CAD build for the part. Positions are in the model's coordinates, mm. A direction names the side the tool comes from. Round coordinates to 2 decimals unless told otherwise and drop trailing zeros. Write each loop counter-clockwise with the first axis right and the second up, starting at its lowest first coordinate (ties: lowest second). Pieces come first, ordered by that corner, then holes. Notation, with made-up numbers: (-6.5, 60) -> (35.5, 60) arc R19 cw to (35.5, 94) -> close; hole circle Ø3 at (12.25, 76). An arc over 180 degrees is marked (long way). Put each result on its own line as item: value. Start each with the question number.
1. Saw through at D-D on x = -4. List the corners of the cut face in (y, z).
2. Flat gauge pins, fed straight in: P1, Ø8, axis at x = -33, y = 33, coming from the -Z side; P2, Ø3, axis at x = 20.5, z = -17.5, coming from the -Y side; P3, Ø12, axis at x = -2.5, y = 25.5, coming from the +Z side. Where does each tip first touch, or does it go through?
3. Saw through at A-A on z = -10.75. List the corners of the cut face in (x, y).
4. Pull direction Z, two halves, no side cores. Call faces 1 (the flat face through (-24, 8, -17)), 2 (the flat face through (30, 32, -2.5)), 3 (the cylindrical face through (23.846, 7.509, -20.944)): pulls with the +Z half, pulls with the -Z half, needs draft (parallel to the pull), parting line crosses it, or undercut.
5. Saw through at C-C on x = -32. State how many separate pieces and enclosed holes the cut face has, and give its area (3 significant figures).
6. 3-axis set-ups, long thin cutter, end or side, ignore diameter. For faces 4 (the flat face through (30, -35, -2.5)), 5 (the flat face through (-31, 30, -22.5)), 6 (the flat face through (30, 32, -22.5)), 7 (the cylindrical face through (-30.237, -29.866, -12.36)): which of +Z, -Z, +X, -X, +Y, -Y reach the whole face in a straight line?
7. Saw through at B-B on y = 10. List the corners of the cut face in (x, z).
8. Drill centre lines: line 1 (Y direction, x = -33, z = -23.1); line 2 (Z direction, x = 36, y = 28). Where is each one in solid material? Low to high. Write a range as from..to.
from build123d import *

# Parameters (mm, degrees)
FRONT_FLANGE_80X80_DEPTH = 2.5
HOUSING_BODY_DEPTH       = 20
REAR_FLANGE_80X80_DEPTH  = 2.5
MOUNTING_HOLES_SKETCH_R  = 3
MOUNTING_HOLES_4X_DEPTH  = 92.5
THROUGH_BORE_SKETCH_50_R = 25
THROUGH_BORE_50_DEPTH    = 132.5
COUNTERBORE_SKETCH_70_R  = 35
COUNTERBORE_70_DEPTH     = 17


with BuildPart() as part:
    # Front Flange Sketch → Front Flange 80x80 (new body)
    with BuildSketch(Plane.XY):
        with BuildLine():
            Line((-33, -40), (33, -40))
            ThreePointArc((33, -40), (37.949747468, -37.949747468), (40, -33))
            Line((40, -33), (40, 33))
            ThreePointArc((40, 33), (37.949747468, 37.949747468), (33, 40))
            Line((33, 40), (-33, 40))
            ThreePointArc((-33, 40), (-37.949747468, 37.949747468), (-40, 33))
            Line((-40, 33), (-40, -33))
            ThreePointArc((-40, -33), (-37.949747468, -37.949747468), (-33, -40))
        make_face()
    extrude(amount=-FRONT_FLANGE_80X80_DEPTH)

    # Housing Body Sketch → Housing Body (add)
    with BuildSketch(Plane(origin=(0, 0, -2.5), x_dir=(-1, 0, 0), z_dir=(0, 0, -1))):
        with BuildLine():
            Line((-14.361406616, 40), (14.361406616, 40))
            ThreePointArc((14.361406616, 40), (30.0520382, 30.0520382), (40, 14.361406616))
            Line((40, 14.361406616), (40, -14.361406616))
            ThreePointArc((40, -14.361406616), (30.0520382, -30.0520382), (14.361406616, -40))
            Line((14.361406616, -40), (-14.361406616, -40))
            ThreePointArc((-14.361406616, -40), (-30.0520382, -30.0520382), (-40, -14.361406616))
            Line((-40, -14.361406616), (-40, 14.361406616))
            ThreePointArc((-40, 14.361406616), (-30.0520382, 30.0520382), (-14.361406616, 40))
        make_face()
    extrude(amount=HOUSING_BODY_DEPTH)

    # Rear Flange Sketch → Rear Flange 80x80 (add)
    with BuildSketch(Plane(origin=(0, 0, -22.5), x_dir=(-1, 0, 0), z_dir=(0, 0, -1))):
        with BuildLine():
            Line((33, -40), (-33, -40))
            ThreePointArc((-33, -40), (-37.949747468, -37.949747468), (-40, -33))
            Line((-40, -33), (-40, 33))
            ThreePointArc((-40, 33), (-37.949747468, 37.949747468), (-33, 40))
            Line((-33, 40), (33, 40))
            ThreePointArc((33, 40), (37.949747468, 37.949747468), (40, 33))
            Line((40, 33), (40, -33))
            ThreePointArc((40, -33), (37.949747468, -37.949747468), (33, -40))
        make_face()
    extrude(amount=REAR_FLANGE_80X80_DEPTH)

    # Mounting Holes Sketch → Mounting Holes 4x (cut)
    with BuildSketch(Plane.XY):
        with Locations(Location((-33, 33, 0), (0, 0, 180))):
            Circle(MOUNTING_HOLES_SKETCH_R)
        with Locations(Location((33, 33, 0), (0, 0, 180))):
            Circle(MOUNTING_HOLES_SKETCH_R)
        with Locations(Location((33, -33, 0), (0, 0, 180))):
            Circle(MOUNTING_HOLES_SKETCH_R)
        with Locations(Location((-33, -33, 0), (0, 0, 180))):
            Circle(MOUNTING_HOLES_SKETCH_R)
    extrude(amount=-MOUNTING_HOLES_4X_DEPTH, mode=Mode.SUBTRACT)

    # Through Bore Sketch Ø50 → Through Bore Ø50 (cut)
    with BuildSketch(Plane.XY):
        Circle(THROUGH_BORE_SKETCH_50_R)
    extrude(amount=-THROUGH_BORE_50_DEPTH, mode=Mode.SUBTRACT)

    # Counterbore Sketch Ø70 → Counterbore Ø70 (cut)
    with BuildSketch(Plane.XY):
        Circle(COUNTERBORE_SKETCH_70_R)
    extrude(amount=-COUNTERBORE_70_DEPTH, mode=Mode.SUBTRACT)


solid = part.part
Return value:
1. outline: (-40, -25) -> (-24.68, -25) -> (-24.68, -17) -> (-34.77, -17) -> (-34.77, 0) -> (-40, 0) -> close; (24.68, -25) -> (40, -25) -> (40, 0) -> (34.77, 0) -> (34.77, -17) -> (24.68, -17) -> close
2. P1: stops at z = -25
2. P2: stops at y = -38.02
2. P3: stops at z = -17
3. outline: (-40, -14.36) arc R42.5 ccw to (-14.36, -40) -> (14.36, -40) arc R42.5 ccw to (40, -14.36) -> (40, 14.36) arc R42.5 ccw to (14.36, 40) -> (-14.36, 40) arc R42.5 ccw to (-40, 14.36) -> close; hole circle Ø70 at (0, 0)
4. face 1: pulls with the +Z half
4. face 2: undercut
4. face 3: needs draft
5. separate pieces: 5
5. enclosed holes: 0
5. area: 980 mm^2
6. face 4: +X, -Y
6. face 5: -X, +Y
6. face 6: +X, +Y
6. face 7: -X, -Y
7. outline: (-40, -25) -> (-22.91, -25) -> (-22.91, -17) -> (-33.54, -17) -> (-33.54, 0) -> (-40, 0) -> close; (22.91, -25) -> (40, -25) -> (40, 0) -> (33.54, 0) -> (33.54, -17) -> (22.91, -17) -> close
8. line 1: y = -40..-36, -30..30, 36..40
8. line 2: z = -25..-22.5, -2.5..0
